Geometry check sheet. Reference: the model listing, model coordinates, mm. Round coordinates to 2 decimals unless told otherwise and drop trailing zeros. Write each loop counter-clockwise with the first axis right and the second up, starting at its lowest first coordinate (ties: lowest second). Pieces come first, ordered by that corner, then holes.
Item 1: Cross-section at C-C (z = 474). Enter the section's corners in (x, y), then the cut area to 3 significant figures.
Item 2: Cross-section at B-B (y = 14). Enter the section's corners in (x, z), then the cut area to 3 significant figures.
Item 3: Depth check by flat-ended pin: P1, Ø8, axis at y = 5, z = 103, coming from the -X side; P2, Ø1.5, axis at y = -23, z = 124.5, coming from the -X side; P3, Ø3, axis at y = 4.5, z = 520.5, coming from the -X side. Enter the tip coordinate at first touch or a pass-through.
Item 4: Cross-section at A-A (x = -6). Enter the section's corners in (y, z).
Item 5: Scan lines: probe 1 along X at (y, z) = (-2.5, 370); probe 2 along Y at (x, z) = (1, 248.5); probe 3 along Y at (x, z) = (3, 58). Record each from-to range of solid material in increasing order.
from build123d import *

# Parameters (mm, degrees)
SKETCH1_R           = 27.5
BOSS_EXTRUDE1_DEPTH = 17.6
SKETCH2_R           = 25
BOSS_EXTRUDE2_DEPTH = 12
SKETCH3_R           = 30
BOSS_EXTRUDE3_DEPTH = 695
SKETCH4_R           = 27.5
BOSS_EXTRUDE4_DEPTH = 17.6
BOSS_EXTRUDE5_START = 12
SKETCH5_R           = 25
BOSS_EXTRUDE5_DEPTH = 12


with BuildPart() as part:
    # Sketch1 → Boss-Extrude1 (new body)
    with BuildSketch(Plane.XY):
        Circle(SKETCH1_R)
    extrude(amount=BOSS_EXTRUDE1_DEPTH)

    # Sketch2 → Boss-Extrude2 (add)
    with BuildSketch(Plane(origin=(0, 0, 0), x_dir=(-1, 0, 0), z_dir=(0, 0, -1))):
        with Locations(Location((0, 0, 0), (0, 0, 180))):
            Circle(SKETCH2_R)
    extrude(amount=BOSS_EXTRUDE2_DEPTH)

    # Sketch3 → Boss-Extrude3 (add)
    with BuildSketch(Plane.XY.offset(17.6)):
        Circle(SKETCH3_R)
    extrude(amount=BOSS_EXTRUDE3_DEPTH)

    # Sketch4 → Boss-Extrude4 (add)
    with BuildSketch(Plane.XY.offset(712.6)):
        Circle(SKETCH4_R)
    extrude(amount=BOSS_EXTRUDE4_DEPTH)

    # Sketch5 → Boss-Extrude5 (add)
    with BuildSketch(Plane.XY.offset(730.2).offset(BOSS_EXTRUDE5_START)):
        Circle(SKETCH5_R)
    extrude(amount=-BOSS_EXTRUDE5_DEPTH)


solid = part.part
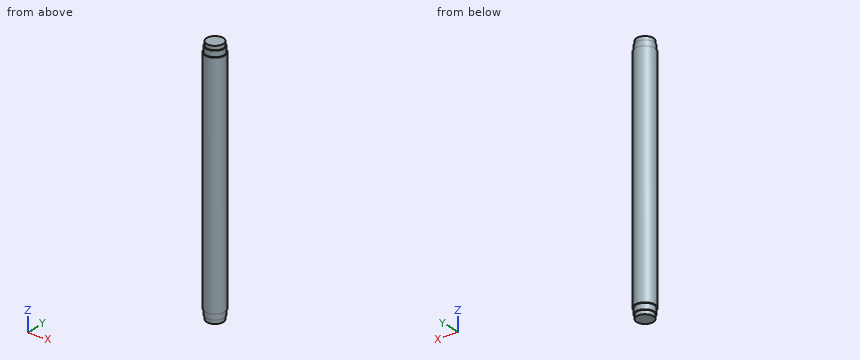
Resolved:
1. outline: circle Ø60 at (0, 0)
1. area: 2,830 mm2
2. outline: (-26.53, 17.6) - (-23.67, 17.6) - (-23.67, 0) - (-20.71, 0) - (-20.71, -12) - (20.71, -12) - (20.71, 0) - (23.67, 0) - (23.67, 17.6) - (26.53, 17.6) - (26.53, 712.6) - (23.67, 712.6) - (23.67, 730.2) - (20.71, 730.2) - (20.71, 742.2) - (-20.71, 742.2) - (-20.71, 730.2) - (-23.67, 730.2) - (-23.67, 712.6) - (-26.53, 712.6) - close
2. area: 39,500 mm2
3. P1: stops at x = -29.98
3. P2: stops at x = -20.12
3. P3: stops at x = -29.85
4. outline: (-29.39, 17.6) - (-26.84, 17.6) - (-26.84, 0) - (-24.27, 0) - (-24.27, -12) - (24.27, -12) - (24.27, 0) - (26.84, 0) - (26.84, 17.6) - (29.39, 17.6) - (29.39, 712.6) - (26.84, 712.6) - (26.84, 730.2) - (24.27, 730.2) - (24.27, 742.2) - (-24.27, 742.2) - (-24.27, 730.2) - (-26.84, 730.2) - (-26.84, 712.6) - (-29.39, 712.6) - close
5. probe 1: x = -29.9 to 29.9
5. probe 2: y = -29.98 to 29.98
5. probe 3: y = -29.85 to 29.85
